The model under review builds one solid part; all positions refer to its coordinate system, in mm. Round coordinates to 2 decimals unless told otherwise and drop trailing zeros. Write each loop counter-clockwise with the first axis right and the second up, starting at its lowest first coordinate (ties: lowest second). Pieces come first, ordered by that corner, then holes. Notation, with made-up numbers: (-3.75, 4) -> (36.25, 4) arc R30 ccw to (36.25, 33) -> close; hole circle Ø8 at (67.5, 54.5). An arc over 180 degrees is marked (long way). Use CSV: the item, a comma, the result in double quotes. Start each with the question number.
1) For pin 1 Ø22.5 at (y, z) = (52.5, 52.5) entering from +X, flat-tipped, find the tip position at first contact; note if it passes through.
2) Wall thickness on probe 1 along Y at (x, z) = (3.5, -61.5); probe 2 along Z at (x, y) = (7.75, 55.5); probe 3 along Y at (x, z) = (6.5, -64.5): over which ranges is each line inside the solid? List them lowest first. Write a range as [from, to].
3) Mouldability with a two-part tool opening along Y and no side actions: class faces 1 (the face through (5, 72.5, 1)), 2 (the face through (5, -70, -70)), 3 (the face through (4.93, -62.8, -58.36)), 4 (the face through (5, -1, 72.5)) as released by +Y, released by -Y, zero draft, split by the parting line, or undercut.
4) Take a section at D-D, the plane y = 52.5. Give the boundary of the cut face in (x, z), then the cut area to 3 significant figures.
5) Take a section at C-C, the plane x = 6. State how many separate pieces and enclosed holes the cut face has, then the cut area to 3 significant figures.
6) Take a section at A-A, the plane y = 12.5. Give the boundary of the cut face in (x, z).
from build123d import *

# Parameters (mm, degrees)
SKETCH_1_W          = 145
SKETCH_1_H          = 145
EXTRUDE_1_DEPTH     = 10
CHAMFER_1_SIZE      = 5
HOLE_WIZARD_M8_1_D  = 6.8
HOLE_WIZARD_M16_1_D = 14
SKETCH_8_R          = 4.5
CUT_EXTRUDE_1_DEPTH = 104.01698889


with BuildPart() as part:
    # 草图1 → 凸台-拉伸1 (new body)
    with BuildSketch(Plane(origin=(0, 0, 0), x_dir=(0, 0, -1), z_dir=(1, 0, 0))):
        Rectangle(SKETCH_1_W, SKETCH_1_H)
    extrude(amount=EXTRUDE_1_DEPTH)

    # 倒角1
    chamfer_1_edges = [part.edges().sort_by_distance(p)[0] for p in [
        (5, -72.5, -72.5),
        (5, -72.5, 72.5),
        (5, 72.5, 72.5),
        (5, 72.5, -72.5),
    ]]
    chamfer(chamfer_1_edges, length=CHAMFER_1_SIZE)

    # M8 螺纹孔1 (through all)
    with Locations(Plane(origin=(10, 0, 0), x_dir=(0, 0, -1), z_dir=(1, 0, 0))):
        with Locations((61.5, -61.5), (2.5, 19.5), (61.5, 19.5), (2.5, -61.5), (-11.5, -61.5), (-11.5, -16.5), (61.5, -16.5)):
            Hole(HOLE_WIZARD_M8_1_D / 2)

    # M16 螺纹孔1 (through all)
    with Locations(Plane(origin=(10, 0, 0), x_dir=(0, 0, -1), z_dir=(1, 0, 0))):
        with Locations((-52.5, 52.5)):
            Hole(HOLE_WIZARD_M16_1_D / 2)

    # 草图8 → 切除-拉伸1 (cut, through all)
    with BuildSketch(Plane(origin=(10, 0, 0), x_dir=(0, 0, -1), z_dir=(1, 0, 0))):
        with Locations((-12.5, 52.5)):
            Circle(SKETCH_8_R)
        with Locations((47.5, 52.5)):
            Circle(SKETCH_8_R)
        with Locations((-52.5, 12.5)):
            Circle(SKETCH_8_R)
        with Locations((-52.5, -47.5)):
            Circle(SKETCH_8_R)
    extrude(amount=-CUT_EXTRUDE_1_DEPTH, mode=Mode.SUBTRACT)


solid = part.part
Values found:
1,pin 1,"x = 10"
2,probe 1,"[-72.5, -64.9], [-58.1, -19.9], [-13.1, 16.1], [22.9, 72.5]"
2,probe 2,"[-72.5, -50.85], [-44.15, 9.15], [15.85, 46.18], [58.82, 72.5]"
2,probe 3,"[-72.5, -63.1], [-59.9, -18.1], [-14.9, 17.9], [21.1, 72.5]"
3,face 1,"released by +Y"
3,face 2,"released by -Y"
3,face 3,"undercut"
3,face 4,"zero draft"
4,outline,"(0, -72.5) -> (10, -72.5) -> (10, -52) -> (0, -52) -> close; (0, -43) -> (10, -43) -> (10, 8) -> (0, 8) -> close; (0, 17) -> (10, 17) -> (10, 45.5) -> (0, 45.5) -> close; (0, 59.5) -> (10, 59.5) -> (10, 72.5) -> (0, 72.5) -> close"
4,area,"1,130 mm²"
5,separate pieces,"1"
5,enclosed holes,"12"
5,area,"20,300 mm²"
6,outline,"(0, -72.5) -> (10, -72.5) -> (10, 48) -> (0, 48) -> close; (0, 57) -> (10, 57) -> (10, 72.5) -> (0, 72.5) -> close"
